from build123d import *


with BuildPart() as part:
    # Sketch1 → Revolve1 (revolve)
    with BuildSketch(Plane.XY, mode=Mode.PRIVATE) as revolve1_sk:
        Polygon((28.5, 3.25), (0, 3.25), (0, 0), (115, 0), (115, 5.5), (99, 5.5), (99, 8), (96, 9), (57, 9), (49, 8), (49, 6), (28.5, 6), align=None)
    revolve(revolve1_sk.sketch.rotate(Axis((115, 0, 0), (-1, 0, 0)), 90), axis=Axis((115, 0, 0), (-1, 0, 0)))


solid = part.part
Source: CAD feature listing. Evaluate the final solid. Frame: model axes, mm. A direction names the side the tool comes from. Give positions to 0.01 mm unless a question says otherwise; leave off trailing zeros. Order: outer loops, then holes, each group sorted by start corner. A loop starts at its lowest first (then second) coordinate and runs counter-clockwise, first axis right, second up. Notation, with made-up numbers: (59, 51.5) -> (65, 51.5) arc R23 ccw to (65, 65.5) -> close; hole circle Ø2 at (81.25, 80.25). An arc over 180 degrees is marked (long way). Write item = value, one per line.
Item 1: Set-up query: faces 1 (the face through (28.5, 3, -3)), 2 (the face through (99, -5.4, 1.7)), 3 (the face through (76.227, -6.083, 6.633)). Return all of +Z, -Z, +X, -X, +Y, -Y with unobstructed straight access to the full face (end or side cutting, diameter ignored); none if empty.
Check result:
face_1 = -X
face_2 = +X
face_3 = +X, -X
Item 2: Section query D-D (x = 58.5). Output: boundary loops of the cut face in (y, z), then the cut area to 3 significant figures.
Check result:
outline = circle Ø18 at (0, 0)
area = 254 mm²
Item 3: Section query A-A (z = 0). Output: boundary loops of the cut face in (x, y), then the cut area to 3 significant figures.
Check result:
outline = (0, -3.25) -> (28.5, -3.25) -> (28.5, -6) -> (49, -6) -> (49, -8) -> (57, -9) -> (96, -9) -> (99, -8) -> (99, -5.5) -> (115, -5.5) -> (115, 5.5) -> (99, 5.5) -> (99, 8) -> (96, 9) -> (57, 9) -> (49, 8) -> (49, 6) -> (28.5, 6) -> (28.5, 3.25) -> (0, 3.25) -> close
area = 1,500 mm²
Item 4: Ray query, probe 1 along Y at (x, z) = (33.5, -0.5); probe 2 along X at (y, z) = (-3.5, 6.25); probe 3 along X at (y, z) = (2, -4.5). Return the intervals inside material, ascending.
Check result:
probe_1 = -5.98 to 5.98
probe_2 = 49 to 99
probe_3 = 28.5 to 115
Item 5: Section query C-C (x = 13.5). Output: boundary loops of the cut face in (y, z), then the cut area to 3 significant figures.
Check result:
outline = circle Ø6.5 at (0, 0)
area = 33.2 mm²
Item 6: Contact query for flat-ended pins moving along their axis: pin 1 (6 mm diameter, centred on x = 16, z = -3, fed in from +Y); pin 2 (10 mm diameter, centred on x = 62.5, z = -5.5, fed in from +Y); pin 3 (4 mm diameter, centred on x = 82, y = 6.5, fed in from +Z). Output: stop coordinate, or through.
Check result:
pin_1 = 3.25
pin_2 = 8.99
pin_3 = 7.79
